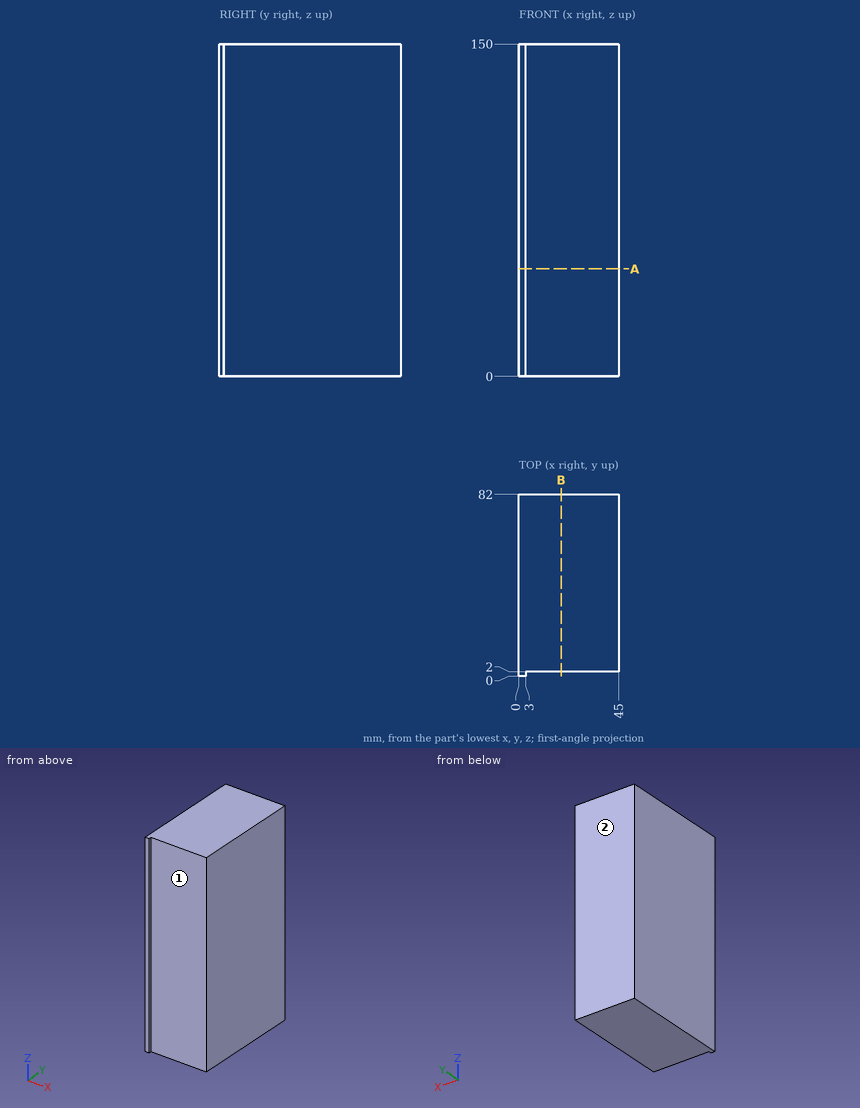
Part print with two shaded views. Sizes in mm from the minimum x, y, z corner. A direction names the side the tool comes from. Coordinates: 2 decimals unless noted, no trailing zeros. Write each loop counter-clockwise with the first axis right and the second up, starting at its lowest first coordinate (ties: lowest second). Pieces come first, ordered by that corner, then holes.
(1) Cut at A-A on z = 48.5. List the corners of the cut face in (x, y), and give its area (3 significant figures).
(2) 3-axis set-ups, long thin cutter, end or side, ignore diameter. For the marked faces 1 and 2: which of +Z, -Z, +X, -X, +Y, -Y reach the whole face in a straight line?
(3) Drill centre line: line 1 (Y direction, x = 27.5, z = 55.5). Where is it in solid material? Low to high.
(4) Pin check, flat tips, straight feed: pin 1 Ø1.6 at (y, z) = (1, 106.5) entering from +X; pin 2 Ø3 at (x, z) = (31, 61.5) entering from -Y; pin 3 Ø12 at (x, y) = (36.5, 41) entering from -Z. Stop position of each tip, or through.
(5) Cut at B-B on x = 19. List the corners of the cut face in (y, z).
Working result:
1. outline: (0, 0) - (3, 0) - (3, 2) - (45, 2) - (45, 82) - (0, 82) - close
1. area: 3,610 mm2
2. face 1: +Z, -Z, +X, -Y
2. face 2: +Z, -Z, +X, -X, +Y
3. line 1: y = 2 to 82
4. pin 1: stops at x = 3
4. pin 2: stops at y = 2
4. pin 3: stops at z = 0
5. outline: (2, 0) - (82, 0) - (82, 150) - (2, 150) - close
